Geometry check sheet. Reference: drawing and pictorial views, mm from the part's lowest x, y, z. Round coordinates to 2 decimals unless told otherwise and drop trailing zeros. Order: outer loops, then holes, each group sorted by start corner. A loop starts at its lowest first (then second) coordinate and runs counter-clockwise, first axis right, second up.
(1) Mould release check, pull along X, two halves, no side actions. Record for the marked faces 1, 2 and 3: released by +X, released by -X, zero draft, split by the parting line, or undercut.
(2) Sectioned sample at C-C, the plane x = 54. Enter the section's corners in (y, z).
(3) Sectioned sample at A-A, the plane z = 17. Enter the section's corners in (x, y).
(4) Thickness scan on probe 1 along X at (y, z) = (80, 1) (1 decimal); probe 2 along Y at (x, z) = (59.5, 17) (1 decimal); probe 3 along Y at (x, z) = (50, 19.25) (1 decimal). Record the ranges inside material, lowest first.
(5) Sectioned sample at B-B, the plane y = 64. Enter the section's corners in (x, z) (1 decimal).
(6) Sectioned sample at D-D, the plane x = 7.5. Enter the section's corners in (y, z) (1 decimal), and give its area (3 significant figures).
(7) Depth check by flat-ended pin: pin 1 (3 mm diameter, centred on x = 47, z = 2.5, fed in from +Y); pin 2 (3 mm diameter, centred on x = 78.5, z = 13.5, fed in from -Y); pin 3 (3 mm diameter, centred on x = 80.5, z = 12, fed in from -Y). Enter the tip coordinate at first touch or a pass-through.
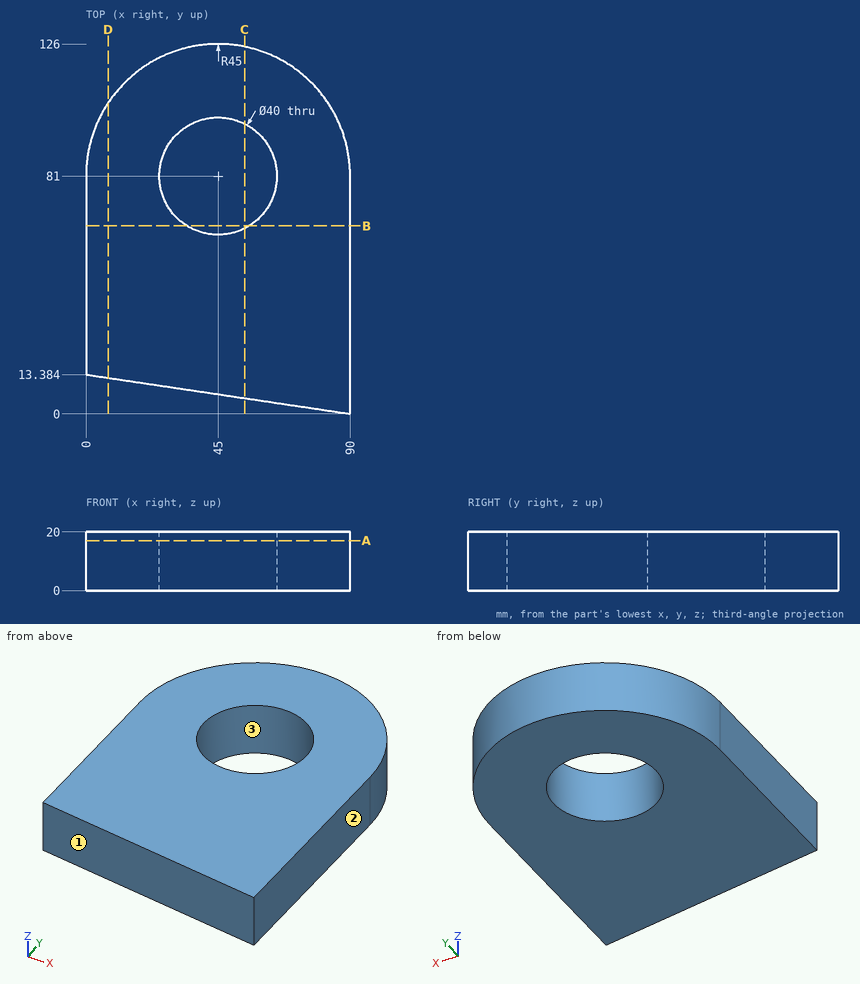
Derived:
1. face 1: released by -X
1. face 2: released by +X
1. face 3: undercut
2. outline: (5.35, 0) - (63.14, 0) - (63.14, 20) - (5.35, 20) - close; (98.86, 0) - (125.09, 0) - (125.09, 20) - (98.86, 20) - close
3. outline: (0, 13.38) - (90, 0) - (90, 81) arc R45 ccw to (0, 81) - close; hole circle Ø40 at (45, 81)
4. probe 1: x = 0 to 25, 65 to 90
4. probe 2: y = 4.5 to 67.2, 94.8 to 123.6
4. probe 3: y = 5.9 to 61.6, 100.4 to 125.7
5. outline: (0, 0) - (34.5, 0) - (34.5, 20) - (0, 20) - close; (55.5, 0) - (90, 0) - (90, 20) - (55.5, 20) - close
6. outline: (12.3, 0) - (105.9, 0) - (105.9, 20) - (12.3, 20) - close
6. area: 1,870 mm2
7. pin 1: stops at y = 126
7. pin 2: stops at y = 1.49
7. pin 3: stops at y = 1.19
